CAD build for the part. Positions are in the model's coordinates, mm. A direction names the side the tool comes from. Round coordinates to 2 decimals unless told otherwise and drop trailing zeros. Loops run counter-clockwise (first coordinate to the right, second up) from the corner with the lowest first, then second, coordinate; pieces in that order, holes last. Notation, with made-up numbers: M 52,74 L 71,74 A34 cw 71,111 Z; hole C 56,73.5 d5. An arc over 180 degrees is marked long. Put each result on its own line as item: value. Start each with the question number.
from build123d import *

# Parameters (mm, degrees)
BASE_BLOCK_SKETCH_W  = 60
BASE_BLOCK_SKETCH_H  = 50
BASE_BLOCK_DEPTH     = 20
UPRIGHT_SKETCH_W     = 10
UPRIGHT_SKETCH_H     = 50
UPRIGHT_DEPTH        = 30
ROUNDED_TOP_SKETCH_R = 25
ROUNDED_TOP_DEPTH    = 10
PIVOT_HOLE_SKETCH_R  = 15
PIVOT_HOLE_DEPTH     = 10
BASE_SLOT_SKETCH_W   = 16
BASE_SLOT_SKETCH_H   = 10
BASE_SLOT_DEPTH      = 50


with BuildPart() as part:
    # Base Block Sketch → Base Block (new body)
    with BuildSketch(Plane(origin=(0, 0, 0), x_dir=(1, 0, 0), z_dir=(0, 1, 0))):
        Rectangle(BASE_BLOCK_SKETCH_W, BASE_BLOCK_SKETCH_H)
    extrude(amount=BASE_BLOCK_DEPTH)

    # Upright Sketch → Upright (add)
    with BuildSketch(Plane(origin=(0, 20, 0), x_dir=(1, 0, 0), z_dir=(0, 1, 0))):
        with Locations((-25, 0)):
            Rectangle(UPRIGHT_SKETCH_W, UPRIGHT_SKETCH_H)
    extrude(amount=UPRIGHT_DEPTH)

    # Rounded Top Sketch → Rounded Top (add)
    with BuildSketch(Plane(origin=(-20, 0, 0), x_dir=(0, 0, -1), z_dir=(1, 0, 0))):
        with Locations((0, 50)):
            Circle(ROUNDED_TOP_SKETCH_R)
    extrude(amount=-ROUNDED_TOP_DEPTH)

    # Pivot Hole Sketch → Pivot Hole (cut)
    with BuildSketch(Plane(origin=(-20, 0, 0), x_dir=(0, 0, -1), z_dir=(1, 0, 0))):
        with Locations((0, 50)):
            Circle(PIVOT_HOLE_SKETCH_R)
    extrude(amount=-PIVOT_HOLE_DEPTH, mode=Mode.SUBTRACT)

    # Base Slot Sketch → Base Slot (cut)
    with BuildSketch(Plane(origin=(30, 0, 0), x_dir=(0, 0, -1), z_dir=(1, 0, 0))):
        with Locations((0, 15)):
            Rectangle(BASE_SLOT_SKETCH_W, BASE_SLOT_SKETCH_H)
    extrude(amount=-BASE_SLOT_DEPTH, mode=Mode.SUBTRACT)


solid = part.part
(1) Cut at D-D on x = -21. List the corners of the cut face in (y, z), and give its area (3 significant figures).
(2) Cut at B-B on x = -7.5. List the corners of the cut face in (y, z), and give its area (3 significant figures).
(3) Tool access for faces 1 (the flat face through (5, 20, 16)), 2 (the cylindrical face through (-24.93, 74.994, -0.55)), 3 (the flat face through (5, 15, 8)): list every direction of +Z, -Z, +X, -X, +Y, -Y with a clear straight run to the whole face (end or side of a thin tool).
(4) Drill centre lines: line 1 along Y through (x, z) = (-22.5, 0); line 2 along Y through (x, z) = (1, -10); line 3 along Y through (x, z) = (-11, -0.5). Where is each one in solid material? Low to high.
(5) Flat gauge pins, fed straight in: pin 1 Ø4 at (x, z) = (7, -17) entering from +Y; pin 2 Ø12 at (x, z) = (-7, 0) entering from +Y; pin 3 Ø15 at (y, z) = (58, -4) entering from +X. Where does each tip first touch, or does it go through?
(6) Cut at A-A on z = 0. List the corners of the cut face in (x, y), and give its area (3 significant figures).
(7) Cut at C-C on y = 52.5. List the corners of the cut face in (x, z), and give its area (3 significant figures).
(8) Mould opens along Y. For faces 4 (the flat face through (5, 15, -8)), 5 (the cylindrical face through (-24.93, 64.872, 1.953)), 6 (the flat face through (5, 20, -17)) say: +Y half, -Y half, draft (parallel to the pull), parting line (faces both ways), or undercut.
Taken from the geometry:
1. outline: M 0,-25 L 50,-25 A25 ccw 50,25 L 0,25 Z; hole C 50,0 d30
1. area: 2,770 mm2
2. outline: M 0,-25 L 20,-25 L 20,-8 L 10,-8 L 10,8 L 20,8 L 20,25 L 0,25 Z
2. area: 840 mm2
3. face 1: +Z, -Z, +X, +Y
3. face 2: +X, -X, +Y
3. face 3: +X, +Y
4. line 1: 0 to 35, 65 to 75
4. line 2: 0 to 20
4. line 3: 0 to 10
5. pin 1: y = 20
5. pin 2: y = 10
5. pin 3: x = -20
6. outline: M -30,0 L 30,0 L 30,10 L -20,10 L -20,35 L -30,35 Z; M -30,65 L -20,65 L -20,75 L -30,75 Z
6. area: 950 mm2
7. outline: M -30,-24.87 L -20,-24.87 L -20,-14.79 L -30,-14.79 Z; M -30,14.79 L -20,14.79 L -20,24.87 L -30,24.87 Z
7. area: 202 mm2
8. face 4: draft
8. face 5: undercut
8. face 6: +Y half
